Geometry check sheet. Reference: the model listing, model coordinates, mm. Face numbers are marked on the shaded views. A direction names the side the tool comes from. Round coordinates to 2 decimals unless told otherwise and drop trailing zeros. Write each loop counter-clockwise with the first axis right and the second up, starting at its lowest first coordinate (ties: lowest second). Pieces come first, ordered by that corner, then holes. Notation, with made-up numbers: M 84,29 L 120,29 A27 cw 120,65 Z; hole C -7,50.5 d5. An arc over 180 degrees is marked long. One line per item, written item: value. Start each with the question number.
1. Scan lines: probe 1 along Y at (x, z) = (-9, 1.5); probe 2 along X at (y, z) = (-1.25, -2). Record each from-to range of solid material in increasing order. Write a range as [from, to].
2. Section check B-B (z = 2.5). Record the boundary of the cut face in (x, y), and give its area (3 significant figures).
3. Access from +Z, -Z, +X, -X, +Y, -Y to the whole of each face (thin tool, end or side, straight path). Record for the marked faces 1 and 2.
4. Section check A-A (x = -16.5). Record the boundary of the cut face in (y, z).
5. Section check C-C (y = -0.5). Record the boundary of the cut face in (x, z), and give its area (3 significant figures).
6. Depth check by flat-ended pin: P1, Ø3, axis at y = 0, z = -0.5, coming from the -X side; P2, Ø1.5, axis at y = -7, z = -2, coming from the +X side. Enter the tip coordinate at first touch or a pass-through.
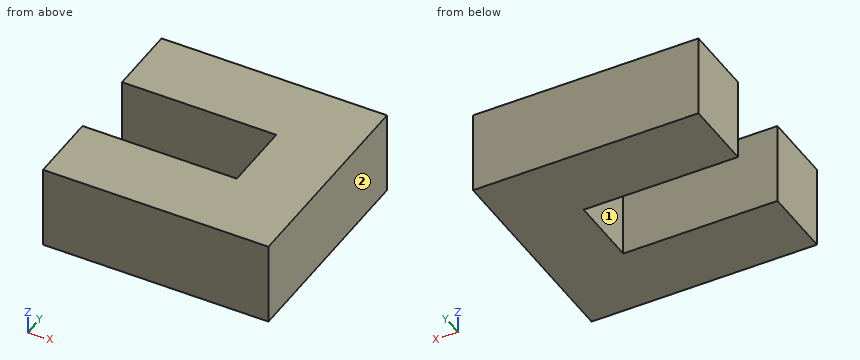
from build123d import *

# Parameters (mm, degrees)
EXTRUDE_1_DEPTH = 3.5


with BuildPart() as part:
    # 草图1 → 凸台-拉伸1 (new, symmetric)
    with BuildSketch(Plane.XY):
        Polygon((0, 0), (0, 9), (-19, 9), (-19, 3), (-6, 3), (-6, -3), (-19, -3), (-19, -9), (0, -9), align=None)
    extrude(amount=EXTRUDE_1_DEPTH, both=True)


solid = part.part
Result sheet:
1. probe 1: y = [-9, -3], [3, 9]
1. probe 2: x = [-6, 0]
2. outline: M -19,-9 L 0,-9 L 0,9 L -19,9 L -19,3 L -6,3 L -6,-3 L -19,-3 Z
2. area: 264 mm2
3. face 1: +Z, -Z, -X
3. face 2: +Z, -Z, +X, +Y, -Y
4. outline: M -9,-3.5 L -3,-3.5 L -3,3.5 L -9,3.5 Z; M 3,-3.5 L 9,-3.5 L 9,3.5 L 3,3.5 Z
5. outline: M -6,-3.5 L 0,-3.5 L 0,3.5 L -6,3.5 Z
5. area: 42.0 mm2
6. P1: stops at x = -6
6. P2: stops at x = 0
